CAD build for the part. Positions are in the model's coordinates, mm. Coordinates: 2 decimals unless noted, no trailing zeros. Loops run counter-clockwise (first coordinate to the right, second up) from the corner with the lowest first, then second, coordinate; pieces in that order, holes last.
1) Saw through at A-A, the plane y = 127.5. Write the cut outline in (x, z), and give its area (4 significant figures).
2) Wall check: line 1 along X through (y, z) = (127.5, 14.5); line 2 along X through (y, z) = (75, 14.25); line 3 along Y through (x, z) = (-765, 12). Give the ranges that are in metal, low to high.
3) Saw through at C-C, the plane z = 10.5. Write the cut outline in (x, y).
4) Pin check, flat tip, straight feed: pin 1 Ø4 at (x, z) = (-113, 14) entering from +Y. Stop position of the tip, or through.
5) Saw through at D-D, the plane x = 59. Write the cut outline in (y, z), and give its area (3 significant figures).
6) Saw through at B-B, the plane x = 765. Write the cut outline in (y, z).
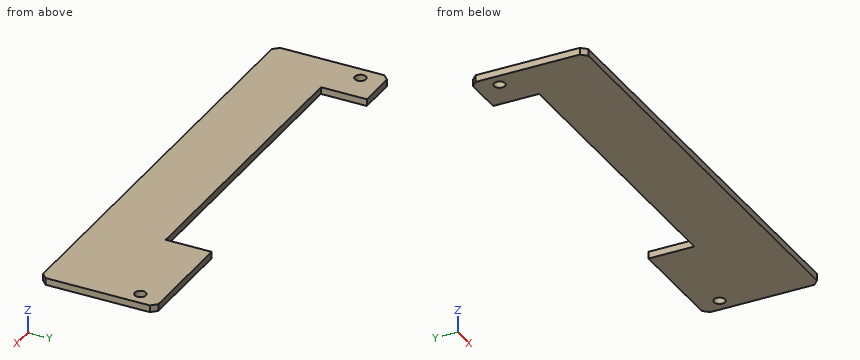
```python
from build123d import *

# Parameters (mm, degrees)
SKETCH1_W               = 1630
SKETCH1_H               = 415
BOSS_EXTRUDE1_DEPTH     = 25
CHAMFER1_SIZE           = 20
CUT_EXTRUDE1_DEPTH      = 842.371647965
CUT_EXTRUDE1_DEPTH_BACK = 842.371647965
SKETCH2_R               = 20
SKETCH2_W               = 1080
SKETCH2_H               = 200


with BuildPart() as part:
    # Sketch1 → Boss-Extrude1 (new body)
    with BuildSketch(Plane.XY):
        Rectangle(SKETCH1_W, SKETCH1_H)
    extrude(amount=BOSS_EXTRUDE1_DEPTH)

    # Chamfer1
    chamfer1_edges = [part.edges().sort_by_distance(p)[0] for p in [
        (-815, 207.5, 12.5),
        (815, 207.5, 12.5),
        (815, -207.5, 12.5),
        (-815, -207.5, 12.5),
    ]]
    chamfer(chamfer1_edges, length=CHAMFER1_SIZE)

    # Sketch2 → Cut-Extrude1 (cut, two sides: drawn at the far end of the back side and taken through both)
    with BuildSketch(Plane.XY.offset(25).offset(-CUT_EXTRUDE1_DEPTH_BACK)):
        with Locations((-765, 127.5)):
            Circle(SKETCH2_R)
        with Locations((765, 127.5)):
            Circle(SKETCH2_R)
        with Locations((-115, 142.5)):
            Rectangle(SKETCH2_W, SKETCH2_H)
    extrude(amount=CUT_EXTRUDE1_DEPTH + CUT_EXTRUDE1_DEPTH_BACK, mode=Mode.SUBTRACT)


solid = part.part
```
Data:
1. outline: (-815, 0) - (-785, 0) - (-785, 25) - (-815, 25) - close; (-745, 0) - (-655, 0) - (-655, 25) - (-745, 25) - close; (425, 0) - (745, 0) - (745, 25) - (425, 25) - close; (785, 0) - (815, 0) - (815, 25) - (785, 25) - close
1. area: 11,750 mm2
2. line 1: x = -815 to -785, -745 to -655, 425 to 745, 785 to 815
2. line 2: x = -815 to -655, 425 to 815
2. line 3: y = -207.5 to 107.5, 147.5 to 207.5
3. outline: (-815, -187.5) - (-795, -207.5) - (795, -207.5) - (815, -187.5) - (815, 187.5) - (795, 207.5) - (425, 207.5) - (425, 42.5) - (-655, 42.5) - (-655, 207.5) - (-795, 207.5) - (-815, 187.5) - close; hole circle Ø40 at (-765, 127.5); hole circle Ø40 at (765, 127.5)
4. pin 1: stops at y = 42.5
5. outline: (-207.5, 0) - (42.5, 0) - (42.5, 25) - (-207.5, 25) - close
5. area: 6,250 mm2
6. outline: (-207.5, 0) - (107.5, 0) - (107.5, 25) - (-207.5, 25) - close; (147.5, 0) - (207.5, 0) - (207.5, 25) - (147.5, 25) - close
